Geometry check sheet. Reference: drawing and pictorial views, mm from the part's lowest x, y, z. A direction names the side the tool comes from. Give positions to 0.01 mm unless a question says otherwise; leave off trailing zeros. Write each loop counter-clockwise with the first axis right and the second up, starting at its lowest first coordinate (ties: lowest second). Pieces come first, ordered by that corner, then holes. Notation, with made-up numbers: M 19.25,61 L 66.25,61 A25 ccw 66.25,97 Z; hole C 25.25,7.25 d6. An arc over 180 degrees is marked long. Write item = value, one per line. Start each with the question number.
1) Cross-section at C-C, the plane x = 65. Record the cut outline in (y, z).
2) Go/stop test with flat-tipped pins: pin 1 (17 mm diameter, centred on x = 68.5, y = 136, fed in from +Z); pin 2 (6 mm diameter, centred on x = 48, z = 43, fed in from +Y); pin 3 (11.5 mm diameter, centred on x = 65, y = 138.5, fed in from -Z). Record where each tip stops, or that it passes through.
3) Cross-section at B-B, the plane y = 139.5. Record the cut outline in (x, z).
4) Access from +Z, -Z, +X, -X, +Y, -Y to the whole of each face (thin tool, end or side, straight path). Record for the marked faces 1, 2, 3, 4 and 5.
5) Cross-section at D-D, the plane z = 106. Record the cut outline in (x, y) (1 decimal).
6) Cross-section at A-A, the plane y = 65. Record the cut outline in (x, z).
7) Scan lines: line 1 along Z through (x, y) = (61.5, 137.5); line 2 along Z through (x, y) = (61.5, 38.5); line 3 along Y through (x, z) = (46.5, 163). Record each from-to range of solid material in increasing order. Write a range as [from, to].
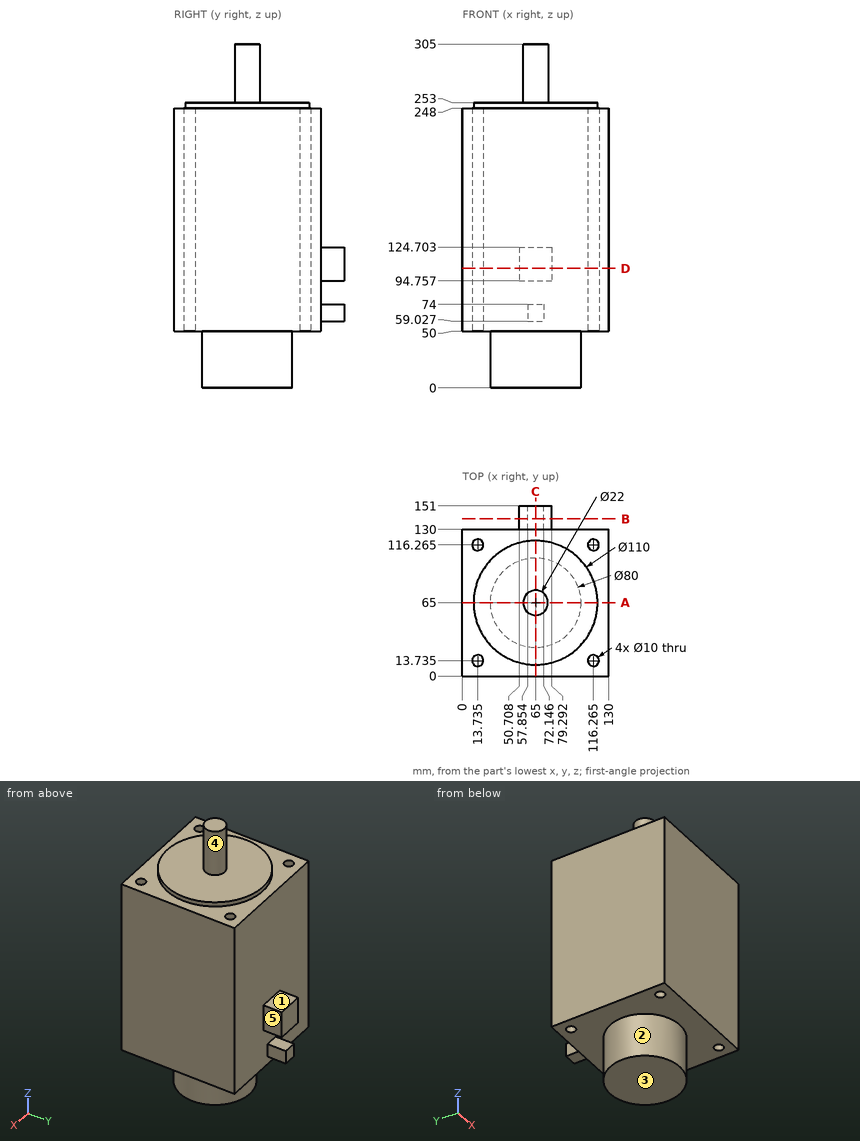
Reply:
q1.outline = M 0,50 L 25,50 L 25,0 L 105,0 L 105,50 L 130,50 L 130,59.03 L 151,59.03 L 151,74 L 130,74 L 130,94.76 L 151,94.76 L 151,124.7 L 130,124.7 L 130,248 L 120,248 L 120,253 L 76,253 L 76,305 L 54,305 L 54,253 L 10,253 L 10,248 L 0,248 Z
q2.pin_1 = 248
q2.pin_2 = 102.47
q2.pin_3 = 59.03
q3.outline = M 50.71,94.76 L 79.29,94.76 L 79.29,124.7 L 50.71,124.7 Z; M 57.85,59.03 L 72.15,59.03 L 72.15,74 L 57.85,74 Z
q4.face_1 = +Z, +X, -X, +Y
q4.face_2 = -Z
q4.face_3 = -Z, +X, -X, +Y, -Y
q4.face_4 = +Z
q4.face_5 = +Z, -Z, +X, +Y
q5.outline = M 0,0 L 130,0 L 130,130 L 79.3,130 L 79.3,151 L 50.7,151 L 50.7,130 L 0,130 Z; hole C 13.7,13.7 d10; hole C 13.7,116.3 d10; hole C 116.3,13.7 d10; hole C 116.3,116.3 d10
q6.outline = M 0,50 L 25,50 L 25,0 L 105,0 L 105,50 L 130,50 L 130,248 L 120,248 L 120,253 L 76,253 L 76,305 L 54,305 L 54,253 L 10,253 L 10,248 L 0,248 Z
q7.line_1 = [59.03, 74], [94.76, 124.7]
q7.line_2 = [0, 253]
q7.line_3 = [0, 130]
